Read the model definition and answer for the solid it produces. Units are mm, in the model's axes. Coordinates: 2 decimals unless noted, no trailing zeros. Write each loop counter-clockwise with the first axis right and the second up, starting at its lowest first coordinate (ties: lowest second). Pieces come first, ordered by that corner, then holes.
(1) Section A-A on x = 214 is taken. Write down the section's boundary in (y, z).
(2) Find the intervals of material crossed by probe 1 along Z at (x, y) = (-38, 1.5); probe 2 along Z at (x, y) = (-68, -2.5); probe 3 along Y at (x, z) = (-304.5, 11), in increasing order.
(3) Section B-B on z = 55 is taken. Write down the section's boundary in (x, y).
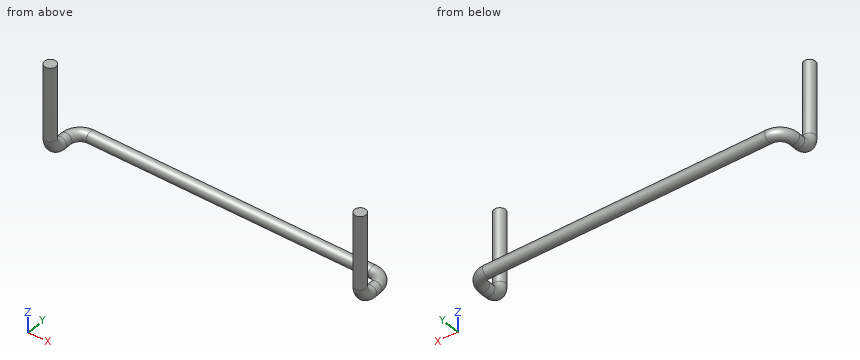
from build123d import *

# Parameters (mm, degrees)
SWEEP1_PROFILE_R = 12.5


with BuildPart() as part:
    # Sweep1: sweep along a curve in space
    with BuildLine() as sweep1_path:
        Line((335, -74.161984871, 30), (335, -74.161984871, 190))
        ThreePointArc((335, -74.161984871, 30), (335, -65.375188307, 8.786796564), (335, -44.161984871, 0))
        Line((335, -30, 0), (335, -44.161984871, 0))
        ThreePointArc((335, -30, 0), (326.213203436, -8.786796564, 0), (305, 0, 0))
        Line((-305, 0, 0), (305, 0, 0))
        ThreePointArc((-305, 0, 0), (-326.213203436, -8.786796564, 0), (-335, -30, 0))
        Line((-335, -30, 0), (-335, -44.161984871, 0))
        ThreePointArc((-335, -74.161984871, 30), (-335, -65.375188307, 8.786796564), (-335, -44.161984871, 0))
        Line((-335, -74.161984871, 30), (-335, -74.161984871, 190))
    # Sweep1 profile (on start of the path) → Sweep1 (sweep)
    with BuildSketch(Plane(origin=(-335, -74.161984871, 190), x_dir=(-1, 0, 0), z_dir=(0, 0, -1))):
        Circle(SWEEP1_PROFILE_R)
    sweep(path=sweep1_path.line)


solid = part.part
Response:
1. outline: circle Ø25 at (0, 0)
2. probe 1: z = -12.41 to 12.41
2. probe 2: z = -12.25 to 12.25
2. probe 3: y = -5.94 to 5.94
3. outline: circle Ø25 at (-335, -74.16); circle Ø25 at (335, -74.16)
